from build123d import *

# Parameters (mm, degrees)
SKETCH_1_W                   = 120
SKETCH_1_H                   = 80
EXTRUDE_1_DEPTH              = 10
CHAMFER_1_SIZE               = 5
HOLE_WIZARD_M5_1_D           = 4.2
HOLE_WIZARD_M5_1_DEPTH       = 14
HOLE_WIZARD_M5_1_CSINK_D     = 5.05
HOLE_WIZARD_M5_1_CSINK_ANGLE = 90
HOLE_WIZARD_M5_1_TIP         = 1.2618073


with BuildPart() as part:
    # 草图1 → 凸台-拉伸1 (new body)
    with BuildSketch(Plane.XY):
        Rectangle(SKETCH_1_W, SKETCH_1_H)
    extrude(amount=EXTRUDE_1_DEPTH)

    # 倒角1
    chamfer_1_edges = [part.edges().sort_by_distance(p)[0] for p in [
        (60, -40, 5),
        (-60, -40, 5),
        (-60, 40, 5),
        (60, 40, 5),
    ]]
    chamfer(chamfer_1_edges, length=CHAMFER_1_SIZE)

    # M5 螺纹孔1
    with Locations(Plane(origin=(0, 20, 10), x_dir=(1, 0, 0), z_dir=(0, 0, 1))):
        with Locations((0, 0), (0, -40)):
            CounterSinkHole(HOLE_WIZARD_M5_1_D / 2, HOLE_WIZARD_M5_1_CSINK_D / 2, depth=HOLE_WIZARD_M5_1_DEPTH, counter_sink_angle=HOLE_WIZARD_M5_1_CSINK_ANGLE)
            with Locations((0, 0, -(HOLE_WIZARD_M5_1_DEPTH + HOLE_WIZARD_M5_1_TIP / 2))):  # 118° drill point
                Cone(0, HOLE_WIZARD_M5_1_D / 2, HOLE_WIZARD_M5_1_TIP, mode=Mode.SUBTRACT)


solid = part.part
Work out the finished part from the listing and answer in its coordinate system (mm). Round coordinates to 2 decimals unless told otherwise and drop trailing zeros. Loops run counter-clockwise (first coordinate to the right, second up) from the corner with the lowest first, then second, coordinate; pieces in that order, holes last. Notation, with made-up numbers: (-35, 52.25) - (15, 52.25) arc R8 cw to (15, 66.25) - close; hole circle Ø10 at (29, 0.5). An arc over 180 degrees is marked (long way). Use one line per item in the form item = value. Start each with the question number.
(1) Determine the mould class of faces 1 (the face through (-57, 38, 5)), 2 (the face through (-1.13, 21.77, 4.72)), 3 (the face through (-1, 1, 10)), 4 (the face through (-1.13, -18.23, 4.72)) for opening direction X: +X half, -X half, draft (parallel to the pull), parting line (faces both ways), or undercut.
(2) A flat-ended cylindrical pin translates along its axis: P1, Ø2.5, axis at x = 0, y = 20, coming from the -Z side. Find the tip coordinate at first contact, or state that the pin passes through.
(3) Find section B-B on y = 20. Determine the outline of the cut face in (x, z) (3 decimals).
(4) Find section A-A on x = 0. Determine the outline of the cut face in (y, z) (3 decimals).
(5) Consider line 1 (Y direction, x = 0, z = 5.25); line 2 (X direction, y = -20, z = 4); line 3 (X direction, y = 19, z = 6). Determine where each line is inside the solid, lowest interval first.
Answer list:
q1.face_1 = -X half
q1.face_2 = undercut
q1.face_3 = draft
q1.face_4 = undercut
q2.P1 = through
q3.outline = (-60, 0) - (-2.1, 0) - (-2.1, 9.575) - (-2.525, 10) - (-60, 10) - close; (2.1, 0) - (60, 0) - (60, 10) - (2.525, 10) - (2.1, 9.575) - close
q4.outline = (-40, 0) - (-22.1, 0) - (-22.1, 9.575) - (-22.525, 10) - (-40, 10) - close; (-17.9, 0) - (17.9, 0) - (17.9, 9.575) - (17.475, 10) - (-17.475, 10) - (-17.9, 9.575) - close; (22.1, 0) - (40, 0) - (40, 10) - (22.525, 10) - (22.1, 9.575) - close
q5.line_1 = -40 to -22.1, -17.9 to 17.9, 22.1 to 40
q5.line_2 = -60 to -2.1, 2.1 to 60
q5.line_3 = -60 to -1.85, 1.85 to 60
